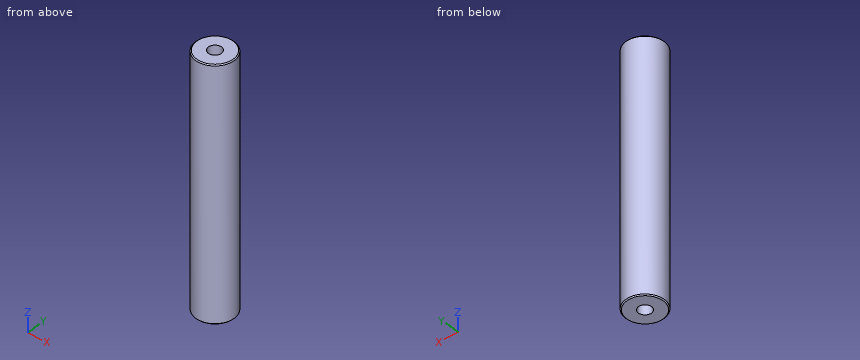
from build123d import *

# Parameters (mm, degrees)
SKETCH_1_R             = 10
EXTRUDE_1_DEPTH        = 130
HOLE_WIZARD_M8_1_D     = 6.8
HOLE_WIZARD_M8_1_DEPTH = 19.75
HOLE_WIZARD_M8_1_TIP   = 2.042926105
HOLE_WIZARD_M8_2_D     = 6.8
HOLE_WIZARD_M8_2_DEPTH = 19.75
HOLE_WIZARD_M8_2_TIP   = 2.042926105
CHAMFER_1_SIZE         = 0.5


with BuildPart() as part:
    # 草图1 → 凸台-拉伸1 (new body)
    with BuildSketch(Plane.XY):
        Circle(SKETCH_1_R)
    extrude(amount=EXTRUDE_1_DEPTH)

    # M8 螺纹孔1
    with Locations(Plane(origin=(0, 0, 0), x_dir=(-1, 0, 0), z_dir=(0, 0, -1))):
        with Locations((0, 0)):
            Hole(HOLE_WIZARD_M8_1_D / 2, depth=HOLE_WIZARD_M8_1_DEPTH)
            with Locations((0, 0, -(HOLE_WIZARD_M8_1_DEPTH + HOLE_WIZARD_M8_1_TIP / 2))):  # 118° drill point
                Cone(0, HOLE_WIZARD_M8_1_D / 2, HOLE_WIZARD_M8_1_TIP, mode=Mode.SUBTRACT)

    # M8 螺纹孔2
    with Locations(Plane.XY.offset(130)):
        with Locations((0, 0)):
            Hole(HOLE_WIZARD_M8_2_D / 2, depth=HOLE_WIZARD_M8_2_DEPTH)
            with Locations((0, 0, -(HOLE_WIZARD_M8_2_DEPTH + HOLE_WIZARD_M8_2_TIP / 2))):  # 118° drill point
                Cone(0, HOLE_WIZARD_M8_2_D / 2, HOLE_WIZARD_M8_2_TIP, mode=Mode.SUBTRACT)

    # 倒角1
    chamfer_1_edges = [part.edges().sort_by_distance(p)[0] for p in [
        (-10, 0, 0),
        (-10, 0, 130),
    ]]
    chamfer(chamfer_1_edges, length=CHAMFER_1_SIZE)


solid = part.part
Geometry check sheet. Reference: the model listing, model coordinates, mm. Round coordinates to 2 decimals unless told otherwise and drop trailing zeros. Order: outer loops, then holes, each group sorted by start corner. A loop starts at its lowest first (then second) coordinate and runs counter-clockwise, first axis right, second up. Notation, with made-up numbers: M 52,71 L 87,71 A33 ccw 87,109 Z; hole C 4.5,-14 d1. An arc over 180 degrees is marked long. Answer in a Markdown table with one row per item. Add a question column.
Item 1: Sectioned sample at B-B, the plane z = 67.5. Enter the section's corners in (x, y), plus the area to 3 significant figures.
Item 2: Material ranges on L1, parallel to Y at x = 0, z = 5.25; L2, parallel to X at y = 8, z = 114; L3, parallel to Y at x = 3.25, z = 28.5, recorded low to high. Write a range as [from, to].
Item 3: Sectioned sample at A-A, the plane z = 13.5. Enter the section's corners in (x, y), plus the area to 3 significant figures.
Item 4: Depth check by flat-ended pin: pin 1 Ø1.5 at (y, z) = (-1, 17) entering from -X; pin 2 Ø4 at (y, z) = (-4, 19.5) entering from -X; pin 3 Ø1.5 at (y, z) = (4.5, 21) entering from -X. Enter the tip coordinate at first touch or a pass-through.
Filled in:
| question | item | result |
|---|---|---|
| 1 | outline | C 0,0 d20 |
| 1 | area | 314 mm² |
| 2 | L1 | y = [-10, -3.4], [3.4, 10] |
| 2 | L2 | x = [-6, 6] |
| 2 | L3 | y = [-9.46, 9.46] |
| 3 | outline | C 0,0 d20; hole C 0,0 d6.8 |
| 3 | area | 278 mm² |
| 4 | pin 1 | stops at x = -10 |
| 4 | pin 2 | stops at x = -9.8 |
| 4 | pin 3 | stops at x = -9.27 |
